from build123d import *

# Parameters (mm, degrees)
SKETCH2_R                       = 7.1501
BOSS_EXTRUDE1_DEPTH             = 106.6292
SKETCH9_R                       = 11.1125
BOSS_EXTRUDE3_DEPTH             = 6.096
CUT_EXTRUDE1_DEPTH              = 49.3776
F_4_48_TAPPED_HOLE1_D           = 2.3749
F_4_48_TAPPED_HOLE1_CSINK_D     = 4.1148
F_4_48_TAPPED_HOLE1_CSINK_ANGLE = 90
SKETCH15_R                      = 7.1374
BOSS_EXTRUDE4_DEPTH             = 65.024
SKETCH16_OUTSIDE_W              = 46.46
SKETCH16_OUTSIDE_H              = 46.46
SKETCH16_OUTSIDE_R              = 7.1374
CUT_EXTRUDE2_DEPTH              = 65.024
CUT_EXTRUDE3_START              = 49.3776
CUT_EXTRUDE3_DEPTH              = 49.3776
SKETCH19_OUTSIDE_W              = 46.46
SKETCH19_OUTSIDE_H              = 46.46
SKETCH19_OUTSIDE_R              = 4.1275
CUT_EXTRUDE4_DEPTH              = 12.7
F_4_48_TAPPED_HOLE2_D           = 2.3749
F_4_48_TAPPED_HOLE2_CSINK_D     = 4.1148
F_4_48_TAPPED_HOLE2_CSINK_ANGLE = 90


with BuildPart() as part:
    # Sketch2 → Boss-Extrude1 (new body)
    with BuildSketch(Plane.XY):
        Circle(SKETCH2_R)
    extrude(amount=-BOSS_EXTRUDE1_DEPTH)

    # Sketch9 → Boss-Extrude3 (add)
    with BuildSketch(Plane.XY.offset(-35.5092)):
        Circle(SKETCH9_R)
    extrude(amount=-BOSS_EXTRUDE3_DEPTH)

    # Sketch11 → Cut-Extrude1 (cut)
    with BuildSketch(Plane(origin=(0, 0, -51.1302), x_dir=(-1, 0, 0), z_dir=(0, 0, -1))):
        with BuildLine():
            Line((-7.110729887, -0.7493), (7.110729887, -0.7493))
            ThreePointArc((7.110729887, -0.7493), (0, 7.1501), (-7.110729887, -0.7493))
        make_face()
    extrude(amount=CUT_EXTRUDE1_DEPTH, mode=Mode.SUBTRACT)

    # #4-48 Tapped Hole1 (through all)
    with Locations(Plane(origin=(0, -0.7493, 0), x_dir=(1, 0, 0), z_dir=(0, 1, 0))):
        with Locations((0, 86.0552), (0, 60.6552)):
            CounterSinkHole(F_4_48_TAPPED_HOLE1_D / 2, F_4_48_TAPPED_HOLE1_CSINK_D / 2, counter_sink_angle=F_4_48_TAPPED_HOLE1_CSINK_ANGLE)

    # Sketch15 → Boss-Extrude4 (add)
    with BuildSketch(Plane(origin=(0, 0, -106.6292), x_dir=(-1, 0, 0), z_dir=(0, 0, -1))):
        Circle(SKETCH15_R)
    extrude(amount=-BOSS_EXTRUDE4_DEPTH)

    # Sketch16 outside → Cut-Extrude2 (cut)
    with BuildSketch(Plane(origin=(0, 0, -106.6292), x_dir=(-1, 0, 0), z_dir=(0, 0, -1))):
        Rectangle(SKETCH16_OUTSIDE_W, SKETCH16_OUTSIDE_H)
        Circle(SKETCH16_OUTSIDE_R, mode=Mode.SUBTRACT)
    extrude(amount=-CUT_EXTRUDE2_DEPTH, mode=Mode.SUBTRACT)

    # Sketch18 → Cut-Extrude3 (cut)
    with BuildSketch(Plane(origin=(0, 0, -51.1302), x_dir=(-1, 0, 0), z_dir=(0, 0, -1)).offset(CUT_EXTRUDE3_START)):
        with BuildLine():
            Line((-7.096607271, -0.762), (7.096607271, -0.762))
            ThreePointArc((7.096607271, -0.762), (0, 7.1374), (-7.096607271, -0.762))
        make_face()
    extrude(amount=-CUT_EXTRUDE3_DEPTH, mode=Mode.SUBTRACT)

    # Sketch19 outside → Cut-Extrude4 (cut)
    with BuildSketch(Plane.XY):
        Rectangle(SKETCH19_OUTSIDE_W, SKETCH19_OUTSIDE_H)
        Circle(SKETCH19_OUTSIDE_R, mode=Mode.SUBTRACT)
    extrude(amount=-CUT_EXTRUDE4_DEPTH, mode=Mode.SUBTRACT)

    # #4-48 Tapped Hole2 (through all)
    with Locations(Plane(origin=(0, -0.762, 0), x_dir=(1, 0, 0), z_dir=(0, 1, 0))):
        with Locations((0, 60.6552), (0, 86.0552)):
            CounterSinkHole(F_4_48_TAPPED_HOLE2_D / 2, F_4_48_TAPPED_HOLE2_CSINK_D / 2, counter_sink_angle=F_4_48_TAPPED_HOLE2_CSINK_ANGLE)


solid = part.part
Could you check a few things on this model? Use its own coordinates, in mm. A direction names the side the tool comes from. Round coordinates to 2 decimals unless told otherwise and drop trailing zeros. Order: outer loops, then holes, each group sorted by start corner. A loop starts at its lowest first (then second) coordinate and runs counter-clockwise, first axis right, second up.
(1) Imagine slicing it at D-D (y = -8.75). Write out the boundary of the cut face in (x, z), plus the area to 3 significant figures.
Response values:
outline: (-6.85, -41.61) - (6.85, -41.61) - (6.85, -35.51) - (-6.85, -35.51) - close
area: 83.5 mm2
(2) Imagine slicing it at C-C (z = -30.5). Write out the boundary of the cut face in (x, y).
Response values:
outline: circle Ø14.3 at (0, 0)
(3) If we mould it in two halves opening along Z, with no side actions, what happens to faces 1 (the flat face through (0, -0.762, -76)), 2 (the flat face through (0, 0, 0)), 3 (the cylindrical face through (10.6, 3.34, -38.51))? For each: released by +Z, released by -Z, zero draft, split by the parting line, or undercut.
Response values:
face 1: undercut
face 2: released by +Z
face 3: zero draft
(4) Imagine slicing it at A-A (x = 0). Count the separate pieces of the cut face and the enclosed holes in it, plus the area to 3 significant figures.
Response values:
separate pieces: 3
enclosed holes: 0
area: 1,070 mm2
(5) Imagine slicing it at B-B (y = 1.25). Write out the boundary of the cut face in (x, z), plus the area to 3 significant figures.
Response values:
outline: (-11.04, -41.61) - (-7.03, -41.61) - (-7.03, -51.13) - (7.03, -51.13) - (7.03, -41.61) - (11.04, -41.61) - (11.04, -35.51) - (7.04, -35.51) - (7.04, -12.7) - (3.93, -12.7) - (3.93, 0) - (-3.93, 0) - (-3.93, -12.7) - (-7.04, -12.7) - (-7.04, -35.51) - (-11.04, -35.51) - close; (-7.03, -106.63) - (7.03, -106.63) - (7.03, -100.51) - (-7.03, -100.51) - close
area: 776 mm2
(6) Please list where these lines run through material, in increasing order: line 1 along Z through (x, y) = (0, -5.9); line 2 along Z through (x, y) = (0, -3.55); line 3 along Z through (x, y) = (-3.5, 3.25).
Response values:
line 1: z = -106.63 to -87.24, -84.87 to -61.84, -59.47 to -12.7
line 2: z = -106.63 to -87.24, -84.87 to -61.84, -59.47 to 0
line 3: z = -106.63 to -100.51, -51.13 to -12.7
(7) Which directions (+Z, -Z, +X, -X, +Y, -Y) give clear straight access to the entire face, cutting with the end or side of a thin tool? Please do faces 4 (the cylindrical face through (-1.55, -6.98, -23.94)), 5 (the flat face through (0, 2, -51.13)), 6 (the cylindrical face through (0.155, -4.424, -61.833)), 7 (the cylindrical face through (1.547, -6.968, -74.572)).
Response values:
face 4: +Z
face 5: +X, -X, +Y
face 6: +Y, -Y
face 7: -Z
(8) I'm going to push flat-ended pins straight in: pin 1 (4 mm diameter, centred on x = 0, z = -60.66, fed in from +Y); pin 2 (10 mm diameter, centred on x = 4.5, z = -74.5, fed in from -Y); pin 3 (2 mm diameter, centred on x = 3.5, z = -59.5, fed in from -Y); pin 4 (1 mm diameter, centred on x = -8, z = -16.5, fed in from +Y). Where does each tip first touch, or does it pass through?
Response values:
pin 1: stops at y = -0.81
pin 2: stops at y = -7.14
pin 3: stops at y = -6.69
pin 4: passes through
